Check sheet for the modelled part. Datum: model origin and axes. Units: mm. A direction names the side the tool comes from. Give positions to 0.01 mm unless a question says otherwise; leave off trailing zeros. Loops run counter-clockwise (first coordinate to the right, second up) from the corner with the lowest first, then second, coordinate; pieces in that order, holes last. Notation, with made-up numbers: (52, 39) -> (56, 39) arc R16 ccw to (56, 65) -> close; hole circle Ø5 at (15.25, -36.5). An arc over 180 degrees is marked (long way). Write each question's results on one line, items separated by ' | '. Start each with the question number.
Item 1: Gauge pin test, flat ends, axial feed: pin 1 Ø4 at (x, z) = (-2, 2) entering from +Y; pin 2 Ø1 at (y, z) = (52.5, 14.5) entering from +X; pin 3 Ø12 at (x, y) = (0, 110) entering from -Z. Record the tip position at first contact, or that the pin passes through.
Item 2: Cross-section at A-A on y = 110. Enter the section's corners in (x, z), then the cut area to 3 significant figures.
Item 3: Access from +Z, -Z, +X, -X, +Y, -Y to the whole of each face (thin tool, end or side, straight path). Record for faces 4 (the face through (0, 5, -11)), 5 (the face through (-6, 350, -4)), 6 (the face through (-1, 60, 4)), 7 (the face through (0, 173, -20)), 8 (the face through (-5.68, 340.14, 2.43)).
Item 4: Cross-section at B-B on z = -14. Enter the section's corners in (x, y), then the cut area to 3 significant figures.
Item 5: Mould release check, pull along Z, two halves, no side actions. Record for faces 1 (the face through (0, 173, 20)), 2 (the face through (4.577, 46.876, 9.951)), 3 (the face through (0, 0, 0)): pulls with the +Z half, pulls with the -Z half, needs draft (parallel to the pull), parting line crosses it, or undercut.
Item 6: Scan lines: line 1 along Y through (x, z) = (0, -13.5); line 2 along X through (y, z) = (340, 15.5); line 3 along Z through (x, y) = (-5, 108.5). Record each from-to range of solid material in increasing order.
from build123d import *

# Parameters (mm, degrees)
SKETCH_1_W                = 20
SKETCH_1_H                = 40
EXTRUDE_1_DEPTH           = 350
SKETCH_2_R                = 6.4
CUT_EXTRUDE_1_DEPTH       = 20
HOLE_WIZARD_M6_1_D        = 5
CHAMFER_1_SIZE            = 1
HOLE_WIZARD_1_D           = 9
HOLE_WIZARD_1_CBORE_D     = 15
HOLE_WIZARD_1_CBORE_DEPTH = 9
HOLE_WIZARD_2_D           = 11
HOLE_WIZARD_2_DEPTH       = 50
HOLE_WIZARD_2_CBORE_D     = 18
HOLE_WIZARD_2_CBORE_DEPTH = 11
HOLE_WIZARD_2_TIP         = 3.304733405


with BuildPart() as part:
    # 草图1 → 凸台-拉伸1 (new body)
    with BuildSketch(Plane(origin=(0, 0, 0), x_dir=(1, 0, 0), z_dir=(0, 1, 0))):
        Rectangle(SKETCH_1_W, SKETCH_1_H)
    extrude(amount=EXTRUDE_1_DEPTH)

    # 草图2 → 切除-拉伸1 (cut)
    with BuildSketch(Plane(origin=(0, 350, 0), x_dir=(1, 0, 0), z_dir=(0, 1, 0))):
        with Locations(Location((0, 0.52, 0), (0, 0, 270))):
            Circle(SKETCH_2_R)
    extrude(amount=-CUT_EXTRUDE_1_DEPTH, mode=Mode.SUBTRACT)

    # M6 螺纹孔1 (through all)
    with Locations(Plane(origin=(0, 0, -20), x_dir=(-1, 0, 0), z_dir=(0, 0, -1))):
        with Locations((0, 340)):
            Hole(HOLE_WIZARD_M6_1_D / 2)

    # 倒角1
    chamfer_1_edges = [part.edges().sort_by_distance(p)[0] for p in [
        (-10, 350, 0),
        (0, 350, 20),
        (10, 350, 0),
        (0, 0, 20),
        (-10, 0, 0),
        (0, 0, -20),
        (10, 0, 0),
        (0, 350, -20),
        (10, 175, 20),
        (-10, 175, 20),
        (-10, 175, -20),
        (10, 175, -20),
    ]]
    chamfer(chamfer_1_edges, length=CHAMFER_1_SIZE)

    # 打孔尺寸(%根据)内六角圆柱头螺钉的类型1 (through all)
    with Locations(Plane(origin=(0, 0, -20), x_dir=(-1, 0, 0), z_dir=(0, 0, -1))):
        with Locations((0, 10), (0, 110)):
            CounterBoreHole(HOLE_WIZARD_1_D / 2, HOLE_WIZARD_1_CBORE_D / 2, HOLE_WIZARD_1_CBORE_DEPTH)

    # 打孔尺寸(%根据)内六角圆柱头螺钉的类型2
    with Locations(Plane(origin=(10, 0, 0), x_dir=(0, 0, -1), z_dir=(1, 0, 0))):
        with Locations((-8, 55.662088154)):
            CounterBoreHole(HOLE_WIZARD_2_D / 2, HOLE_WIZARD_2_CBORE_D / 2, HOLE_WIZARD_2_CBORE_DEPTH, depth=HOLE_WIZARD_2_DEPTH)
            with Locations((0, 0, -(HOLE_WIZARD_2_DEPTH + HOLE_WIZARD_2_TIP / 2))):  # 118° drill point
                Cone(0, HOLE_WIZARD_2_D / 2, HOLE_WIZARD_2_TIP, mode=Mode.SUBTRACT)


solid = part.part
Answer sheet:
1) pin 1: stops at y = 330 | pin 2: stops at x = -1 | pin 3: stops at z = -11
2) outline: (-10, -19) -> (-9, -20) -> (-7.5, -20) -> (-7.5, -11) -> (-4.5, -11) -> (-4.5, 20) -> (-9, 20) -> (-10, 19) -> close; (4.5, -11) -> (7.5, -11) -> (7.5, -20) -> (9, -20) -> (10, -19) -> (10, 19) -> (9, 20) -> (4.5, 20) -> close | area: 384 mm²
3) face 4: -Z | face 5: +Z, -Z, +X, -X, +Y | face 6: +X | face 7: -Z, +X, -X, +Y, -Y | face 8: +Y
4) outline: (-10, 1) -> (-9, 0) -> (9, 0) -> (10, 1) -> (10, 349) -> (9, 350) -> (-9, 350) -> (-10, 349) -> close; hole circle Ø15 at (0, 10); hole circle Ø15 at (0, 110); hole circle Ø5 at (0, 340) | area: 6,620 mm²
5) face 1: pulls with the +Z half | face 2: undercut | face 3: needs draft
6) line 1: y = 0 to 2.5, 17.5 to 102.5, 117.5 to 337.5, 342.5 to 350 | line 2: x = -10 to -2.5, 2.5 to 10 | line 3: z = -11 to 20
